```python
from build123d import *

# Parameters (mm, degrees)
SKETCH_1_W             = 75
SKETCH_1_H             = 32
EXTRUDE_1_DEPTH        = 8
SKETCH_3_W             = 32
SKETCH_3_H             = 24
CUT_EXTRUDE_1_DEPTH    = 44.797830997
HOLE_WIZARD_M6_1_D     = 5
CHAMFER_1_SIZE         = 2
HOLE_WIZARD_M8_1_D     = 6.8
HOLE_WIZARD_M8_1_DEPTH = 19.75
HOLE_WIZARD_M8_1_TIP   = 2.042926105
CHAMFER_2_SIZE         = 2


with BuildPart() as part:
    # 草图1 → 凸台-拉伸1 (new, symmetric)
    with BuildSketch(Plane.XY):
        Rectangle(SKETCH_1_W, SKETCH_1_H)
    extrude(amount=EXTRUDE_1_DEPTH, both=True)

    # 草图3 → 切除-拉伸1 (cut, through all)
    with BuildSketch(Plane.XY.offset(8)):
        with Locations((0, -4)):
            Rectangle(SKETCH_3_W, SKETCH_3_H)
    extrude(amount=-CUT_EXTRUDE_1_DEPTH, mode=Mode.SUBTRACT)

    # M6 螺纹孔1 (through all)
    with Locations(Plane(origin=(37.5, 0, 0), x_dir=(0, 0, -1), z_dir=(1, 0, 0))):
        with Locations((0, -9.5)):
            Hole(HOLE_WIZARD_M6_1_D / 2)

    # 倒角1
    chamfer_1_edges = [part.edges().sort_by_distance(p)[0] for p in [
        (-37.5, 16, 0),
        (37.5, 16, 0),
    ]]
    chamfer(chamfer_1_edges, length=CHAMFER_1_SIZE)

    # M8 螺纹孔1
    with Locations(Plane(origin=(0, 16, 0), x_dir=(1, 0, 0), z_dir=(0, 1, 0))):
        with Locations((-27.5, 0), (27.5, 0)):
            Hole(HOLE_WIZARD_M8_1_D / 2, depth=HOLE_WIZARD_M8_1_DEPTH)
            with Locations((0, 0, -(HOLE_WIZARD_M8_1_DEPTH + HOLE_WIZARD_M8_1_TIP / 2))):  # 118° drill point
                Cone(0, HOLE_WIZARD_M8_1_D / 2, HOLE_WIZARD_M8_1_TIP, mode=Mode.SUBTRACT)

    # 倒角2
    chamfer_2_edges = [part.edges().sort_by_distance(p)[0] for p in [
        (37.5, -16, 0),
        (-37.5, -16, 0),
    ]]
    chamfer(chamfer_2_edges, length=CHAMFER_2_SIZE)


solid = part.part
```
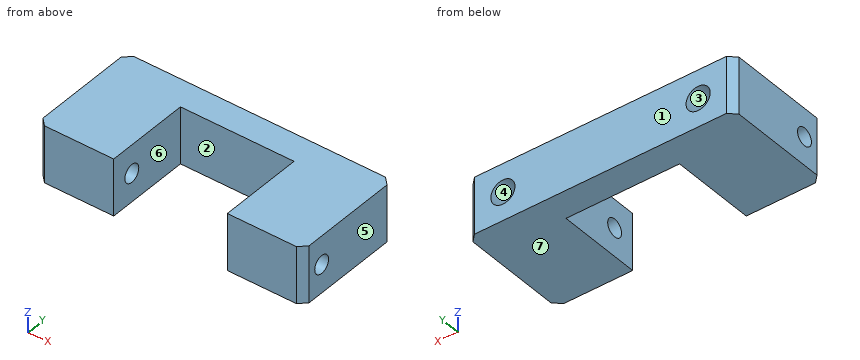
Work out the finished part from the listing and answer in its coordinate system (mm). Face numbers are marked on the shaded views. A direction names the side the tool comes from. Give positions to 0.01 mm unless a question says otherwise; leave off trailing zeros. Loops run counter-clockwise (first coordinate to the right, second up) from the corner with the lowest first, then second, coordinate; pieces in that order, holes last. Notation, with made-up numbers: M 8,58.5 L 57,58.5 A21 cw 57,85.5 Z; hole C 12,69.5 d8. An arc over 180 degrees is marked long. One line per item, written item: value. Start each with the question number.
1. Determine the mould class of the marked faces 4, 5, 6 and 7 for opening direction X: released by +X, released by -X, zero draft, split by the parting line, or undercut.
2. Find section D-D (z = 7.25). Give the vertices of the cut face in (x, y), and give its area (3 significant figures).
3. Find section C-C (x = 17.5). Give the vertices of the cut face in (y, z).
4. Find section B-B (y = -9.5). Give the vertices of the cut face in (x, z), and give its area (3 significant figures).
5. Find the intervals of material crossed by probe 1 along Z at (x, y) = (-27.5, 5); probe 2 along X at (y, z) = (6.5, 2); probe 3 along X at (y, z) = (-3.5, -2.5), in increasing order.
6. This flat-tipped pin is pushed along its axis until it touches: P1, Ø3, axis at x = 15.5, z = 2.5, coming from the -Y side. Where does it stop, or does it pass through?
7. Which of the six approach directions +Z, -Z, +X, -X, +Y, -Y give full straight-line access (tool end or side, diameter ignored) to the marked faces 1, 2 and 3?
8. Find section A-A (y = -2.5). Give the vertices of the cut face in (x, z).
Reported:
1. face 4: undercut
1. face 5: released by +X
1. face 6: undercut
1. face 7: zero draft
2. outline: M -37.5,-14 L -35.5,-16 L -16,-16 L -16,8 L 16,8 L 16,-16 L 35.5,-16 L 37.5,-14 L 37.5,14 L 35.5,16 L -35.5,16 L -37.5,14 Z
2. area: 1,620 mm²
3. outline: M -16,-8 L 16,-8 L 16,8 L -16,8 Z; hole C -9.5,0 d5
4. outline: M -37.5,-8 L -16,-8 L -16,-2.5 L -37.5,-2.5 Z; M -37.5,2.5 L -16,2.5 L -16,8 L -37.5,8 Z; M 16,-8 L 37.5,-8 L 37.5,-2.5 L 16,-2.5 Z; M 16,2.5 L 37.5,2.5 L 37.5,8 L 16,8 Z
4. area: 473 mm²
5. probe 1: z = -8 to -3.4, 3.4 to 8
5. probe 2: x = -37.5 to -30.25, -24.75 to -16, 16 to 24.75, 30.25 to 37.5
5. probe 3: x = -37.5 to -29.8, -25.2 to -16, 16 to 25.2, 29.8 to 37.5
6. P1: stops at y = -16
7. face 1: +Z, -Z, +X, -X, +Y
7. face 2: +Z, -Z, -Y
7. face 3: +Y
8. outline: M -37.5,-8 L -16,-8 L -16,8 L -37.5,8 Z; M 16,-8 L 37.5,-8 L 37.5,8 L 16,8 Z; hole C -27.5,0 d6.8; hole C 27.5,0 d6.8
